```python
from build123d import *

# Parameters (mm, degrees)
CUT_EXTRUDE_1_DEPTH      = 970.651483782
CUT_EXTRUDE_1_DEPTH_BACK = 970.651483782
SKETCH_2_R               = 20
SKETCH_3_W               = 28.175076561
SKETCH_3_H               = 100
CUT_EXTRUDE_2_DEPTH      = 885.810149128


with BuildPart() as part:
    # Sketch 1 → Revolve 1 (revolve)
    with BuildSketch(Plane.XY, mode=Mode.PRIVATE) as revolve_1_sk:
        Polygon((0, 40), (-883, 40), (-883, 35), (-968, 35), (-968, 0), (-750, 0), (-750, 22.5), (0, 22.5), align=None)
    revolve(revolve_1_sk.sketch.rotate(Axis((-802.16755253, 0, 0), (1, 0, 0)), 90), axis=Axis((-802.16755253, 0, 0), (1, 0, 0)))

    # Sketch 2 → Cut-Extrude 1 (cut, two sides: drawn at the far end of the back side and taken through both)
    with BuildSketch(Plane.XY.offset(-CUT_EXTRUDE_1_DEPTH_BACK)):
        with BuildLine():
            Line((-968, 35), (-968, 0))
            ThreePointArc((-968, 0), (-957.748737342, 24.748737342), (-933, 35))
            Line((-933, 35), (-968, 35))
        make_face()
        with BuildLine():
            Line((-968, 0), (-968, -35))
            Line((-968, -35), (-933, -35))
            ThreePointArc((-933, -35), (-957.748737342, -24.748737342), (-968, 0))
        make_face()
        with Locations((-933, 0)):
            Circle(SKETCH_2_R)
    extrude(amount=CUT_EXTRUDE_1_DEPTH + CUT_EXTRUDE_1_DEPTH_BACK, mode=Mode.SUBTRACT)

    # Sketch 3 → Cut-Extrude 2 (cut, through all)
    with BuildSketch(Plane.ZY.offset(883)):
        with Locations((-36.58753828, 0)):
            Rectangle(SKETCH_3_W, SKETCH_3_H)
        with Locations((36.58753828, 0)):
            Rectangle(SKETCH_3_W, SKETCH_3_H)
    extrude(amount=CUT_EXTRUDE_2_DEPTH, mode=Mode.SUBTRACT)


solid = part.part
```
For this review, take the finished solid that the model builds, in its own axes (mm). A direction names the side the tool comes from. Round coordinates to 2 decimals unless told otherwise and drop trailing zeros. Write each loop counter-clockwise with the first axis right and the second up, starting at its lowest first coordinate (ties: lowest second). Pieces come first, ordered by that corner, then holes. Notation, with made-up numbers: (86, 89) - (96, 89) arc R23 ccw to (96, 126) - close; hole circle Ø9 at (-12, 18.25). An arc over 180 degrees is marked (long way). Write each question's results on one line, items separated by ' | '.
Item 1: For faces 1 (the face through (-912, -35, 0)), 2 (the face through (-369.75, 19.961, 10.382)), 3 (the face through (-912, 35, 0)), 4 (the face through (-915, 12, 22.5)), list the 3-axis set-ups (+Z, -Z, +X, -X, +Y, -Y) from which the entire face can be reached by the end or side of a thin tool; tool diameter is ignored.
Calculated:
face 1: -X, -Y | face 2: +X | face 3: -X, +Y | face 4: +Z, -X, +Y, -Y
Item 2: Take a section at B-B on x = -325.5. State the section outline as (y, z) points, then the cut area to 3 significant figures.
Calculated:
outline: circle Ø80 at (0, 0); hole circle Ø45 at (0, 0) | area: 3,440 mm^2
Item 3: Draft analysis for pull direction X (two halves, no side actions). For faces 5 (the face through (-750, 0, 0)), 6 (the face through (-915, -12, -22.5)), 7 (the face through (-913.924, 6.007, -0.315)), state which applies: pulls with the +X half, pulls with the -X half, needs draft (parallel to the pull), parting line crosses it, or undercut.
Calculated:
face 5: pulls with the +X half | face 6: needs draft | face 7: undercut
Item 4: Take a section at C-C on y = -9.5. State the section outline as (x, z) points, then the cut area to 3 significant figures.
Calculated:
outline: (-966.69, -22.5) - (-950.6, -22.5) - (-950.6, 22.5) - (-966.69, 22.5) - close; (-915.4, -22.5) - (-883, -22.5) - (-883, -38.86) - (0, -38.86) - (0, -20.4) - (-750, -20.4) - (-750, 20.4) - (0, 20.4) - (0, 38.86) - (-883, 38.86) - (-883, 22.5) - (-915.4, 22.5) - close | area: 40,200 mm^2
Item 5: To check wall thickness, follow line 1 along Y through (x, z) = (-198, 0); line 2 along Z through (x, y) = (-144, -18); line 3 along Z through (x, y) = (-551, 15). State the ranges of each line that lie inside material, in increasing order. Write a range as from..to.
Calculated:
line 1: y = -40..-22.5, 22.5..40 | line 2: z = -35.72..-13.5, 13.5..35.72 | line 3: z = -37.08..-16.77, 16.77..37.08
Item 6: For pin 1 (2 mm diameter, centred on x = -312, z = 26.5, fed in from -Y); pin 2 (10 mm diameter, centred on y = 26, z = -14.5, fed in from -X); pin 3 (3 mm diameter, centred on y = -14, z = -2.5, fed in from -X), all flat-tipped, find the tip position at first contact; note any pin that passes through.
Calculated:
pin 1: stops at y = -30.82 | pin 2: stops at x = -961 | pin 3: stops at x = -965.69
Item 7: Take a section at A-A on z = 0. State the section outline as (x, y) points, then the cut area to 3 significant figures.
Calculated:
outline: (-933, -35) - (-883, -35) - (-883, -40) - (0, -40) - (0, -22.5) - (-750, -22.5) - (-750, 22.5) - (0, 22.5) - (0, 40) - (-883, 40) - (-883, 35) - (-933, 35) arc R35 ccw to start; hole circle Ø40 at (-933, 0) | area: 41,100 mm^2
